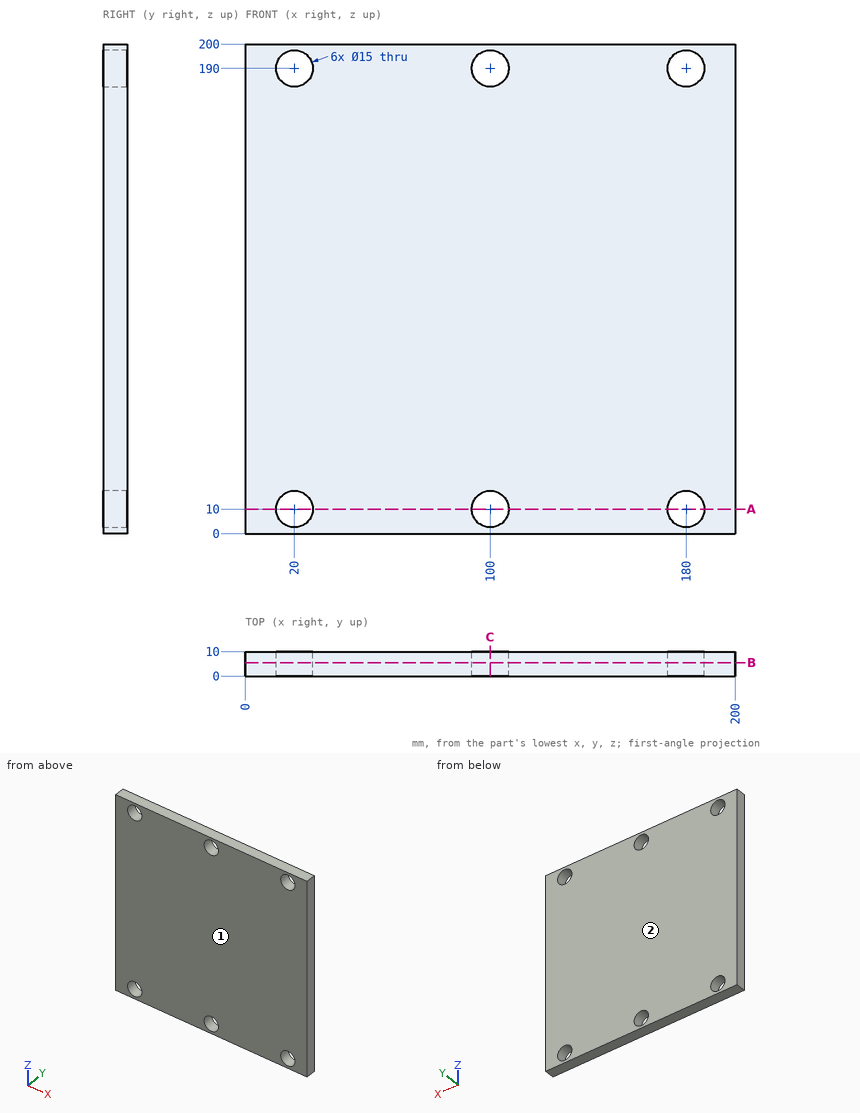
Here's the drawing with two shaded views (mm, measured from the low corner). I have some questions. Coordinates: 2 decimals unless noted, no trailing zeros. Write each loop counter-clockwise with the first axis right and the second up, starting at its lowest first coordinate (ties: lowest second). Pieces come first, ordered by that corner, then holes. Notation, with made-up numbers: (60.5, 7) - (70.5, 7) arc R9 ccw to (70.5, 19) - close; hole circle Ø2 at (-27, -18.5). An arc over 180 degrees is marked (long way). Return JSON: item names as keys, results as strings.
Q1. If we section it at C-C (x = 100): Please give me the cut outline in (y, z), then the cut area to 3 significant figures.
Computed values:
{"outline": "(0, 0) - (10, 0) - (10, 2.5) - (0, 2.5) - close; (0, 17.5) - (10, 17.5) - (10, 182.5) - (0, 182.5) - close; (0, 197.5) - (10, 197.5) - (10, 200) - (0, 200) - close", "area": "1,700 mm2"}
Q2. Thinking about a two-plate mould opening in Y: for the marked faces 1 and 2, which applies, +Y half, -Y half, draft (parallel to the pull), parting line (faces both ways), or undercut?
Computed values:
{"face 1": "-Y half", "face 2": "+Y half"}
Q3. If we section it at A-A (z = 10): Please give me the cut outline in (x, y), then the cut area to 3 significant figures.
Computed values:
{"outline": "(0, 0) - (12.5, 0) - (12.5, 10) - (0, 10) - close; (27.5, 0) - (92.5, 0) - (92.5, 10) - (27.5, 10) - close; (107.5, 0) - (172.5, 0) - (172.5, 10) - (107.5, 10) - close; (187.5, 0) - (200, 0) - (200, 10) - (187.5, 10) - close", "area": "1,550 mm2"}
Q4. Please list where this line runs through material, in increasing order: L1, parallel to X at y = 2.5, z = 190. Write a range as from..to.
Computed values:
{"L1": "x = 0..12.5, 27.5..92.5, 107.5..172.5, 187.5..200"}
Q5. If we section it at B-B (y = 5.5): Please give me the cut outline in (x, z), then the cut area to 3 significant figures.
Computed values:
{"outline": "(0, 0) - (200, 0) - (200, 200) - (0, 200) - close; hole circle Ø15 at (20, 10); hole circle Ø15 at (20, 190); hole circle Ø15 at (100, 10); hole circle Ø15 at (100, 190); hole circle Ø15 at (180, 10); hole circle Ø15 at (180, 190)", "area": "38,900 mm2"}
